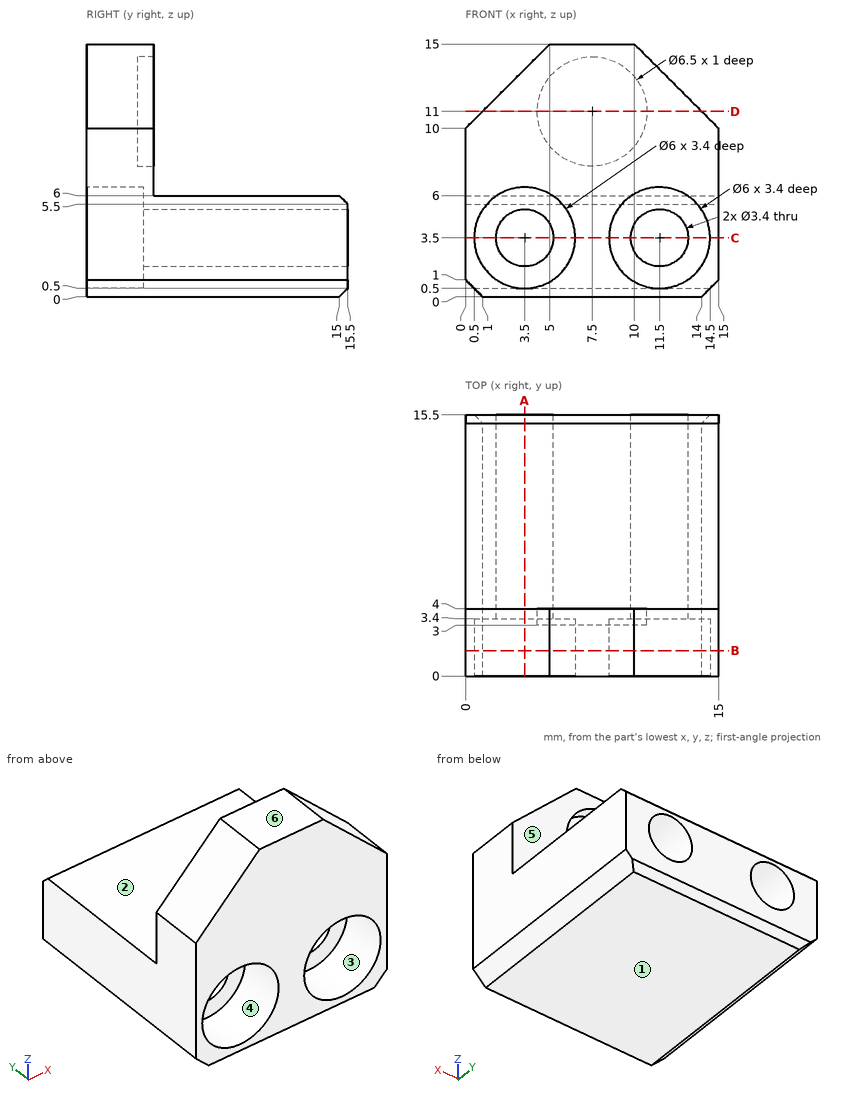
Geometry check sheet. Reference: drawing and pictorial views, mm from the part's lowest x, y, z. A direction names the side the tool comes from. Round coordinates to 2 decimals unless told otherwise and drop trailing zeros. Write each loop counter-clockwise with the first axis right and the second up, starting at its lowest first coordinate (ties: lowest second). Pieces come first, ordered by that corner, then holes.
1. Section check D-D on z = 11. Enter the section's corners in (x, y), plus the area to 3 significant figures.
2. Section check C-C on z = 3.5. Enter the section's corners in (x, y), plus the area to 3 significant figures.
3. Gauge pin test, flat ends, axial feed: P1, Ø3, axis at x = 4, z = 12.5, coming from the +Y side; P2, Ø2, axis at x = 7.5, z = 10, coming from the +Y side; P3, Ø3.5, axis at x = 11.5, z = 3.5, coming from the -Y side. Record the tip position at first contact, or that the pin passes through.
4. Scan lines: L1, parallel to X at y = 3.4, z = 11; L2, parallel to X at y = 11, z = 3.25; L3, parallel to Y at x = 5.75, z = 7.5. Record each from-to range of solid material in increasing order.
5. Draft check along Z on the marked faces 3, 4, 5 and 6. Enter one of: +Z half, -Z half, draft (parallel to the pull), parting line (faces both ways), or undercut.
6. Access from +Z, -Z, +X, -X, +Y, -Y to the whole of each face (thin tool, end or side, straight path). Record for the marked faces 1 and 2.
7. Section check B-B on y = 1.5. Enter the section's corners in (x, z).
8. Section check A-A on x = 3.5. Enter the section's corners in (y, z), plus the area to 3 significant figures.
Answer:
1. outline: (1, 0) - (14, 0) - (14, 4) - (10.75, 4) - (10.75, 3) - (4.25, 3) - (4.25, 4) - (1, 4) - close
1. area: 45.5 mm2
2. outline: (0, 0) - (0.5, 0) - (0.5, 3.4) - (1.8, 3.4) - (1.8, 15.5) - (0, 15.5) - close; (5.2, 3.4) - (6.5, 3.4) - (6.5, 0) - (8.5, 0) - (8.5, 3.4) - (9.8, 3.4) - (9.8, 15.5) - (5.2, 15.5) - close; (13.2, 3.4) - (14.5, 3.4) - (14.5, 0) - (15, 0) - (15, 15.5) - (13.2, 15.5) - close
2. area: 109 mm2
3. P1: stops at y = 4
3. P2: stops at y = 3
3. P3: stops at y = 3.4
4. L1: x = 1 to 4.25, 10.75 to 14
4. L2: x = 0 to 1.82, 5.18 to 9.82, 13.18 to 15
4. L3: y = 0 to 4
5. face 3: undercut
5. face 4: undercut
5. face 5: draft
5. face 6: +Z half
6. face 1: -Z, +X, -X, +Y, -Y
6. face 2: +Z, +X, -X, +Y
7. outline: (0, 1) - (1, 0) - (14, 0) - (15, 1) - (15, 10) - (10, 15) - (5, 15) - (0, 10) - close; hole circle Ø6 at (3.5, 3.5); hole circle Ø6 at (11.5, 3.5)
8. outline: (0, 0) - (15, 0) - (15.5, 0.5) - (15.5, 1.8) - (3.4, 1.8) - (3.4, 0.5) - (0, 0.5) - close; (0, 6.5) - (3.4, 6.5) - (3.4, 5.2) - (15.5, 5.2) - (15.5, 5.5) - (15, 6) - (4, 6) - (4, 13.5) - (0, 13.5) - close
8. area: 61.2 mm2
